Job drawing, mm, ordinate dimensions from the low corner. One solid piece. A direction names the side the tool comes from. Give positions to 0.01 mm unless a question says otherwise; leave off trailing zeros. Order: outer loops, then holes, each group sorted by start corner. A loop starts at its lowest first (then second) coordinate and runs counter-clockwise, first axis right, second up. Notation, with made-up numbers: (46, -20) -> (102, -20) arc R12 ccw to (102, -4) -> close; hole circle Ø11 at (-23, 71). An arc over 180 degrees is marked (long way). Use CSV: the item, a comma, the result in double quotes. Start each with the question number.
1. 3-axis set-ups, long thin cutter, end or side, ignore diameter. For the marked faces 1 and 2: which of +Z, -Z, +X, -X, +Y, -Y reach the whole face in a straight line?
2. Wall check: line 1 (X direction, y = 16, z = 56). Give the ranges that are in metal, low to high. Write a range as from..to.
3. Cut at B-B on z = 65.5. List the corners of the cut face in (x, y).
4. Pull direction Y, two halves, no side cores. Call the marked faces 3, 4 and 5: released by +Y, released by -Y, zero draft, split by the parting line, or undercut.
5. Cut at A-A on y = 32. List the corners of the cut face in (x, z), then the cut area to 3 significant figures.
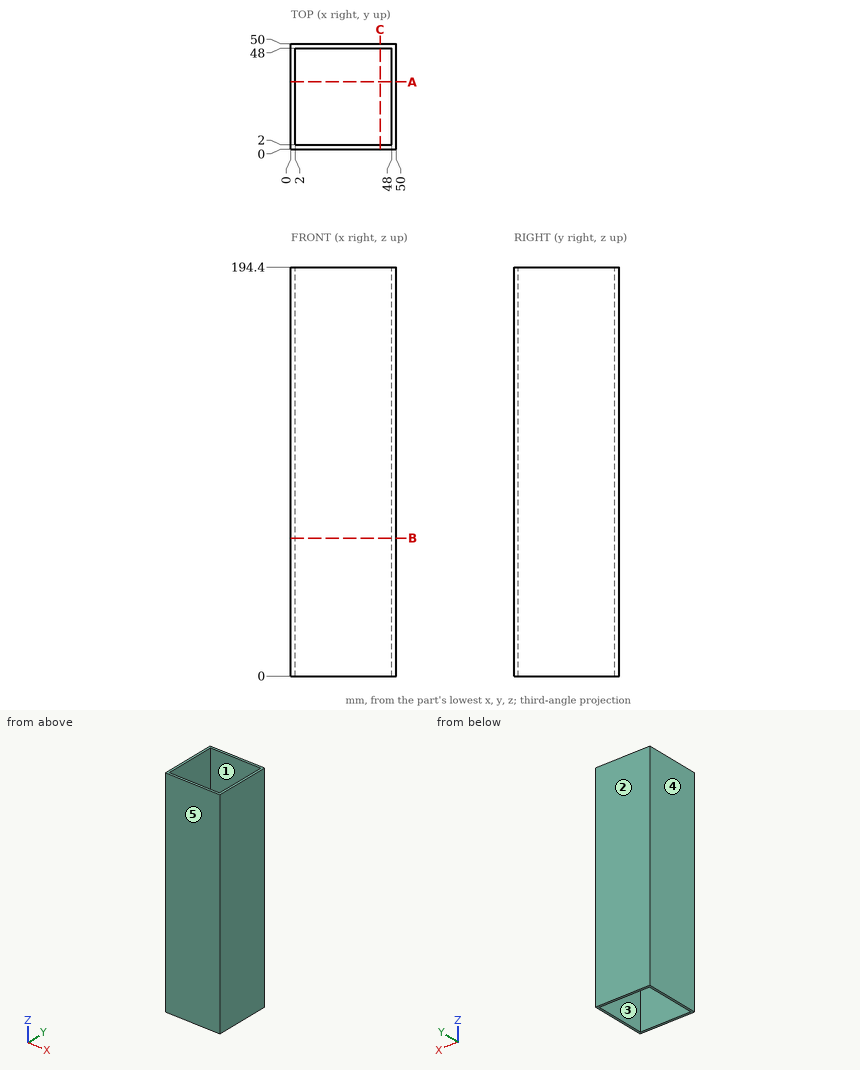
Verdict:
1,face 1,"+Z, -Z"
1,face 2,"+Z, -Z, +X, -X, +Y"
2,line 1,"0..2, 48..50"
3,outline,"(0, 0) -> (50, 0) -> (50, 50) -> (0, 50) -> close; hole (2, 2) -> (48, 2) -> (48, 48) -> (2, 48) -> close"
4,face 3,"undercut"
4,face 4,"zero draft"
4,face 5,"released by -Y"
5,outline,"(0, 0) -> (2, 0) -> (2, 194.4) -> (0, 194.4) -> close; (48, 0) -> (50, 0) -> (50, 194.4) -> (48, 194.4) -> close"
5,area,"778 mm^2"
